```python
from build123d import *

# Parameters (mm, degrees)
HEX_BODY_22MM_DEPTH       = 22
SPIGOT_SKETCH_11_R        = 5.5
SPIGOT_11X8_DEPTH         = 8
SPIGOT_BORE_SKETCH_R      = 4
SPIGOT_THROUGH_BORE_DEPTH = 33.276152187
HEX_BORE_SKETCH_12_R      = 6
HEX_BORE_12X15_DEPTH      = 15


with BuildPart() as part:
    # Hex Profile Sketch → Hex Body 22mm (new body)
    with BuildSketch(Plane.XY):
        Polygon((9, 0), (4.5, 7.794228634), (-4.5, 7.794228634), (-9, 0), (-4.5, -7.794228634), (4.5, -7.794228634), align=None)
    extrude(amount=HEX_BODY_22MM_DEPTH)

    # Spigot Sketch Ø11 → Spigot Ø11x8 (add)
    with BuildSketch(Plane.XY.offset(22)):
        Circle(SPIGOT_SKETCH_11_R)
    extrude(amount=SPIGOT_11X8_DEPTH)

    # Spigot Bore Sketch → Spigot Through Bore (cut, through all)
    with BuildSketch(Plane.XY.offset(30)):
        Circle(SPIGOT_BORE_SKETCH_R)
    extrude(amount=-SPIGOT_THROUGH_BORE_DEPTH, mode=Mode.SUBTRACT)

    # Hex Bore Sketch Ø12 → Hex Bore Ø12x15 (cut)
    with BuildSketch(Plane(origin=(0, 0, 0), x_dir=(-1, 0, 0), z_dir=(0, 0, -1))):
        Circle(HEX_BORE_SKETCH_12_R)
    extrude(amount=-HEX_BORE_12X15_DEPTH, mode=Mode.SUBTRACT)


solid = part.part
```
Input: part model. Units: mm. Frame: model coordinates. A direction names the side the tool comes from. Coordinates: 2 decimals unless noted, no trailing zeros. Write each loop counter-clockwise with the first axis right and the second up, starting at its lowest first coordinate (ties: lowest second). Pieces come first, ordered by that corner, then holes.
1) Section D-D on z = 4.25. Output: boundary loops of the cut face in (x, y).
2) Section C-C on y = 1. Output: boundary loops of the cut face in (x, z).
3) Pin query (flat end, axial travel): pin 1 Ø2 at (y, z) = (5.5, 9.5) entering from +X; pin 2 Ø3 at (y, z) = (-3, 21) entering from +X; pin 3 Ø2 at (x, y) = (-1.5, -5.5) entering from +Z; pin 4 Ø5 at (y, z) = (-3, 10) entering from +X. Return the tip coordinate at first contact, or that it passes through.
4) Section B-B on z = 18. Output: boundary loops of the cut face in (x, y), and give its area (3 significant figures).
5) Mould query, pull axis Y, two halves, no side actions, for faces 1 (the cylindrical face through (-1.19, -5.37, 25.94)), 2 (the cylindrical face through (-0.867, -3.905, 22.605)), 3 (the flat face through (-6.72, 3.95, 10.85)). Classes: pulls with the +Y half, pulls with the -Y half, needs draft (parallel to the pull), parting line crosses it, or undercut.
6) Material intervals for line 1 along Y through (x, z) = (0, 4.5); line 2 along Z through (x, y) = (-5.75, 3.75); line 3 along Y through (x, z) = (0, 27), sorted ascending.
7) Set-up query: faces 4 (the flat face through (1.42, -3.92, 15)), 5 (the flat face through (0, -7.794, 11)), 6 (the flat face through (6, 0, 22)). Return all of +Z, -Z, +X, -X, +Y, -Y with unobstructed straight access to the full face (end or side cutting, diameter ignored); none if empty.
8) Section A-A on x = 0. Output: boundary loops of the cut face in (y, z), and give its area (3 significant figures).
Check result:
1. outline: (-9, 0) - (-4.5, -7.79) - (4.5, -7.79) - (9, 0) - (4.5, 7.79) - (-4.5, 7.79) - close; hole circle Ø12 at (0, 0)
2. outline: (-8.42, 0) - (-5.92, 0) - (-5.92, 15) - (-3.87, 15) - (-3.87, 30) - (-5.41, 30) - (-5.41, 22) - (-8.42, 22) - close; (3.87, 15) - (5.92, 15) - (5.92, 0) - (8.42, 0) - (8.42, 22) - (5.41, 22) - (5.41, 30) - (3.87, 30) - close
3. pin 1: stops at x = 6.4
3. pin 2: stops at x = 8.13
3. pin 3: stops at z = 30
3. pin 4: stops at x = 8.71
4. outline: (-9, 0) - (-4.5, -7.79) - (4.5, -7.79) - (9, 0) - (4.5, 7.79) - (-4.5, 7.79) - close; hole circle Ø8 at (0, 0)
4. area: 160 mm2
5. face 1: parting line crosses it
5. face 2: undercut
5. face 3: pulls with the +Y half
6. line 1: y = -7.79 to -6, 6 to 7.79
6. line 2: z = 0 to 22
6. line 3: y = -5.5 to -4, 4 to 5.5
7. face 4: -Z
7. face 5: +Z, -Z, +X, -X, -Y
7. face 6: +Z
8. outline: (-7.79, 0) - (-6, 0) - (-6, 15) - (-4, 15) - (-4, 30) - (-5.5, 30) - (-5.5, 22) - (-7.79, 22) - close; (4, 15) - (6, 15) - (6, 0) - (7.79, 0) - (7.79, 22) - (5.5, 22) - (5.5, 30) - (4, 30) - close
8. area: 131 mm2
